```python
from build123d import *

# Parameters (mm, degrees)
CUT_EXTRUDE1_DEPTH      = 62.057369758
CUT_EXTRUDE1_DEPTH_BACK = 62.057369758


with BuildPart() as part:
    # Sweep2: sweep along a path in Dimension sketch
    with BuildLine(Plane.XY) as sweep2_path:
        Line((56.7, 2.95), (6.7, 2.95))
        ThreePointArc((6.7, 2.95), (5.417163248, 3.21991314), (4.351858935, 3.983883006))
        ThreePointArc((4.351858935, 3.983883006), (-5.9, 0), (4.351858935, -3.983883006))
        ThreePointArc((4.351858935, -3.983883006), (5.417163248, -3.21991314), (6.7, -2.95))
        Line((6.7, -2.95), (60.7, -2.95))
    # Sketch2 → Sweep2 (sweep)
    with BuildSketch(Plane(origin=(56.7, 2.95, 0), x_dir=(0, 0, 1), z_dir=(-1, 0, 0))):
        with BuildLine():
            Line((-2.949983051, -2.94), (2.949983051, -2.94))
            ThreePointArc((2.949983051, -2.94), (0, 0), (-2.949983051, -2.94))
        make_face()
    sweep(path=sweep2_path.line)

    # Sketch3 → Cut-Extrude1 (cut, two sides: drawn at the far end of the back side and taken through both)
    with BuildSketch(Plane.XY.offset(-CUT_EXTRUDE1_DEPTH_BACK)):
        Polygon((56.7, 1.47), (54.596982728, 2.95), (60.71, 2.95), (60.71, -2.95), (58.589980652, -2.95), (60.7, -1.48), (58.596982728, 0), (54.589980652, 0), align=None)
    extrude(amount=CUT_EXTRUDE1_DEPTH + CUT_EXTRUDE1_DEPTH_BACK, mode=Mode.SUBTRACT)


solid = part.part
```
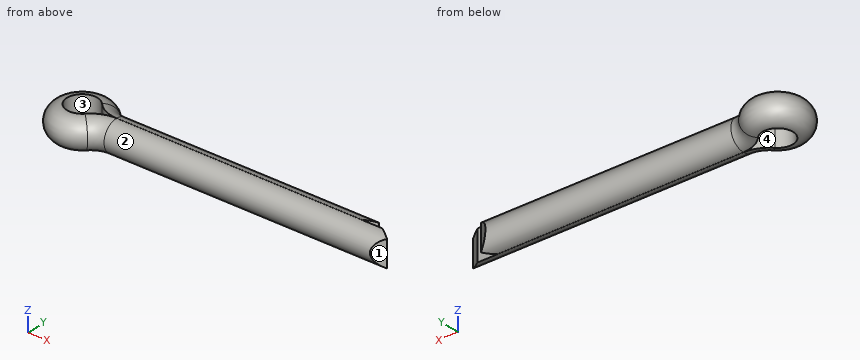
Here's how the part is built. I have some questions about the finished solid (model axes, mm). Face numbers are marked on the shaded views. Give positions to 0.01 mm unless a question says otherwise; leave off trailing zeros. Write each loop counter-clockwise with the first axis right and the second up, starting at its lowest first coordinate (ties: lowest second). Pieces come first, ordered by that corner, then holes.
(1) If I drill on L1, parallel to Y at x = 0, z = 0.2; L2, parallel to Z at x = -2.5, y = -2; L3, parallel to X at y = -1, z = -2.35, over which ranges is the centre line in solid material (lowest first)?
Output values:
L1: y = -5.89 to -2.96, 2.96 to 5.89
L2: z = -2.94 to 2.94
L3: x = -4.63 to -2.79, 3.36 to 60.02
(2) Imagine slicing it at A-A, the plane x = 52.5. Write out the boundary of the cut face in (y, z), and give its area (3 significant figures).
Output values:
outline: (-0.01, -2.95) - (-0.01, 2.95) arc R2.95 ccw to start; (0.01, -2.95) arc R2.95 ccw to (0.01, 2.95) - close
area: 27.2 mm2
(3) Will these pins go through, and if not, where does the flat tip stop? pin 1 (2 mm diameter, centred on x = 34.5, z = 1, fed in from +Y); pin 2 (1.5 mm diameter, centred on x = 31, z = 0.5, fed in from -Y).
Output values:
pin 1: stops at y = 2.95
pin 2: stops at y = -2.95
(4) Thinking about a two-plate mould opening in X: for the marked faces 1, 2, 3 and 4, which applies, pulls with the +X half, pulls with the -X half, needs draft (parallel to the pull), parting line crosses it, or undercut?
Output values:
face 1: pulls with the +X half
face 2: needs draft
face 3: undercut
face 4: undercut
